from build123d import *

# Parameters (mm, degrees)
DISC_PROFILE_115_R      = 57.5
DISC_115X15_DEPTH       = 15
HOLES_4X_15_SKETCH_R    = 7.5
HOLES_4X_15_ON_80_DEPTH = 15
CENTRE_BORE_32_SKETCH_R = 16
CENTRE_BORE_32_DEPTH    = 15
RIM_START               = -15
RIM_NOTCHES_DEPTH       = 15


with BuildPart() as part:
    # Disc Profile Ø115 → Disc Ø115x15 (new body)
    with BuildSketch(Plane.XY):
        Circle(DISC_PROFILE_115_R)
    extrude(amount=DISC_115X15_DEPTH)

    # Holes 4xØ15 Sketch → Holes 4xØ15 on Ø80 (cut)
    with BuildSketch(Plane.XY.offset(15)):
        with Locations((34.641016151, 20)):
            Circle(HOLES_4X_15_SKETCH_R)
        with Locations((0, -40)):
            Circle(HOLES_4X_15_SKETCH_R)
        with Locations((-34.641016151, 20)):
            Circle(HOLES_4X_15_SKETCH_R)
    extrude(amount=-HOLES_4X_15_ON_80_DEPTH, mode=Mode.SUBTRACT)

    # Centre Bore Ø32 Sketch → Centre Bore Ø32 (cut)
    with BuildSketch(Plane.XY.offset(15)):
        Circle(CENTRE_BORE_32_SKETCH_R)
    extrude(amount=-CENTRE_BORE_32_DEPTH, mode=Mode.SUBTRACT)

    # Rim Notches Sketch → Rim Notches (cut)
    with BuildSketch(Plane.XY.offset(15).offset(RIM_START)):
        with BuildLine():
            Line((-5, 49.282196187), (5, 49.282196187))
            Line((5, 49.282196187), (5, 57.282196187))
            ThreePointArc((5, 57.282196187), (0, 57.5), (-5, 57.282196187))
            Line((-5, 57.282196187), (-5, 49.282196187))
        make_face()
        with BuildLine():
            Line((45.179633852, -20.310971075), (40.179633852, -28.971225112))
            Line((40.179633852, -28.971225112), (47.107837082, -32.971225112))
            ThreePointArc((47.107837082, -32.971225112), (49.796460718, -28.75), (52.107837082, -24.310971075))
            Line((52.107837082, -24.310971075), (45.179633852, -20.310971075))
        make_face()
        with BuildLine():
            Line((-40.179633852, -28.971225112), (-45.179633852, -20.310971075))
            Line((-45.179633852, -20.310971075), (-52.107837082, -24.310971075))
            ThreePointArc((-52.107837082, -24.310971075), (-49.796460718, -28.75), (-47.107837082, -32.971225112))
            Line((-47.107837082, -32.971225112), (-40.179633852, -28.971225112))
        make_face()
    extrude(amount=RIM_NOTCHES_DEPTH, mode=Mode.SUBTRACT)


solid = part.part
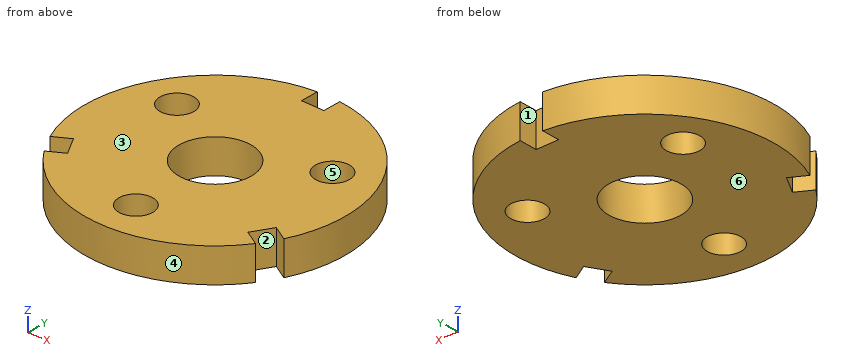
Verification items for the finished model (mm, model axes). Face numbers are marked on the shaded views. A direction names the side the tool comes from. Give positions to 0.01 mm unless a question says otherwise; leave off trailing zeros. Order: outer loops, then holes, each group sorted by start corner. A loop starts at its lowest first (then second) coordinate and runs counter-clockwise, first axis right, second up. Notation, with made-up numbers: M 58,10.5 L 68,10.5 A22 ccw 68,45.5 Z; hole C 75.25,-10.75 d5. An arc over 180 degrees is marked long. Answer as a JSON object with one key per item and string values. Group by question number.
1) Scan lines: line 1 along Y through (x, z) = (0, 10.5); line 2 along X through (y, z) = (-5, 4.75); line 3 along X through (y, z) = (11, 6.75). Record each from-to range of solid material in increasing order. Write a range as [from, to].
2) Cross-section at C-C (z = 10). Enter the section's corners in (x, y).
3) Depth check by flat-ended pin: pin 1 Ø2 at (x, z) = (43.5, 5) entering from +Y; pin 2 Ø6 at (y, z) = (14, 7.5) entering from -X; pin 3 Ø1 at (x, z) = (-25, 9) entering from +Y. Enter the tip coordinate at first touch or a pass-through.
4) Mould release check, pull along X, two halves, no side actions. Record for the marked faces 4, 5 and 6: released by +X, released by -X, zero draft, split by the parting line, or undercut.
5) Cross-section at A-A (y = 0). Enter the section's corners in (x, z), then the cut area to 4 significant figures.
6) Cross-section at D-D (y = 25). Enter the section's corners in (x, z), then the cut area to 3 significant figures.
7) Access from +Z, -Z, +X, -X, +Y, -Y to the whole of each face (thin tool, end or side, straight path). Record for the marked faces 1, 2 and 3.
8) Cross-section at B-B (x = 0). Enter the section's corners in (y, z).
Result sheet:
{
 "1": {"line 1": "y = [-57.5, -47.5], [-32.5, -16], [16, 49.28]", "line 2": "x = [-57.28, -15.2], [15.2, 57.28]", "line 3": "x = [-56.44, -11.62], [11.62, 56.44]"},
 "2": {"outline": "M -52.11,-24.31 L -45.18,-20.31 L -40.18,-28.97 L -47.11,-32.97 A57.5 ccw 47.11,-32.97 L 40.18,-28.97 L 45.18,-20.31 L 52.11,-24.31 A57.5 ccw 5,57.28 L 5,49.28 L -5,49.28 L -5,57.28 A57.5 ccw Z; hole C -34.64,20 d15; hole C 0,0 d32; hole C 0,-40 d15; hole C 34.64,20 d15"},
 "3": {"pin 1": "stops at y = 38.73", "pin 2": "stops at x = -56.44", "pin 3": "stops at y = 52.02"},
 "4": {"face 4": "split by the parting line", "face 5": "undercut", "face 6": "zero draft"},
 "5": {"outline": "M -57.5,0 L -16,0 L -16,15 L -57.5,15 Z; M 16,0 L 57.5,0 L 57.5,15 L 16,15 Z", "area": "1,245 mm2"},
 "6": {"outline": "M -51.78,0 L -40.23,0 L -40.23,15 L -51.78,15 Z; M -29.05,0 L 29.05,0 L 29.05,15 L -29.05,15 Z; M 40.23,0 L 51.78,0 L 51.78,15 L 40.23,15 Z", "area": "1,220 mm2"},
 "7": {"face 1": "+Z, -Z, +Y", "face 2": "+Z, -Z", "face 3": "+Z, +X, -X, +Y, -Y"},
 "8": {"outline": "M -57.5,0 L -47.5,0 L -47.5,15 L -57.5,15 Z; M -32.5,0 L -16,0 L -16,15 L -32.5,15 Z; M 16,0 L 49.28,0 L 49.28,15 L 16,15 Z"}
}
